from build123d import *

# Parameters (mm, degrees)
EXTRUDE_1_DEPTH           = 4
HOLE_WIZARD_1_D           = 3.4
HOLE_WIZARD_1_CBORE_D     = 6.5
HOLE_WIZARD_1_CBORE_DEPTH = 3.4
HOLE_WIZARD_M3_1_D        = 2.5
HOLE_WIZARD_M4_1_D        = 3.3
CHAMFER_1_SIZE            = 0.5


with BuildPart() as part:
    # 草图1 → 凸台-拉伸1 (new, symmetric)
    with BuildSketch(Plane(origin=(0, 0, 0), x_dir=(0, 0, -1), z_dir=(1, 0, 0))):
        with BuildLine():
            Line((20.5, -5), (-20.5, -5))
            ThreePointArc((-20.5, -5), (-25.5, 0), (-20.5, 5))
            Line((-20.5, 5), (20.5, 5))
            ThreePointArc((20.5, 5), (25.5, 0), (20.5, -5))
        make_face()
    extrude(amount=EXTRUDE_1_DEPTH, both=True)

    # 打孔尺寸(%根据)内六角圆柱头螺钉的类型1 (through all)
    with Locations(Plane(origin=(4, 0, 0), x_dir=(0, 0, -1), z_dir=(1, 0, 0))):
        with Locations((-20.5, 0)):
            CounterBoreHole(HOLE_WIZARD_1_D / 2, HOLE_WIZARD_1_CBORE_D / 2, HOLE_WIZARD_1_CBORE_DEPTH)

    # M3 螺纹孔1 (through all)
    with Locations(Plane(origin=(4, 0, 0), x_dir=(0, 0, -1), z_dir=(1, 0, 0))):
        with Locations((-4.5, 0)):
            Hole(HOLE_WIZARD_M3_1_D / 2)

    # M4 螺纹孔1 (through all)
    with Locations(Plane(origin=(4, 0, 0), x_dir=(0, 0, -1), z_dir=(1, 0, 0))):
        with Locations((20.5, 0)):
            Hole(HOLE_WIZARD_M4_1_D / 2)

    # 倒角1
    chamfer_1_edges = [part.edges().sort_by_distance(p)[0] for p in [
        (4, 0, 25.5),
        (4, -5, 0),
        (4, 0, -25.5),
        (-4, -5, 0),
        (-4, 0, 25.5),
        (-4, 5, 0),
        (-4, 0, -25.5),
        (4, 5, 0),
    ]]
    chamfer(chamfer_1_edges, length=CHAMFER_1_SIZE)


solid = part.part
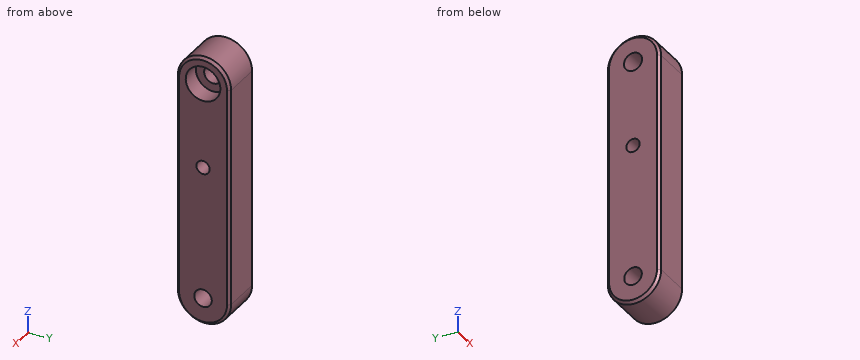
Source: CAD feature listing. Evaluate the final solid. Frame: model axes, mm. Give positions to 0.01 mm unless a question says otherwise; leave off trailing zeros. Order: outer loops, then holes, each group sorted by start corner. A loop starts at its lowest first (then second) coordinate and runs counter-clockwise, first axis right, second up. Notation, with made-up numbers: (-15.5, -26.75) -> (15.5, -26.75) arc R6 cw to (15.5, -16.75) -> close; hole circle Ø11 at (-25, 14). An arc over 180 degrees is marked (long way). Write item = value, one per line.
Q1. Cut plane A-A, the plane y = 0. Output: boundary loops of the cut face in (x, z).
Data:
outline = (-4, -25) -> (-3.5, -25.5) -> (3.5, -25.5) -> (4, -25) -> (4, -22.15) -> (-4, -22.15) -> close; (-4, -18.85) -> (4, -18.85) -> (4, 3.25) -> (-4, 3.25) -> close; (-4, 5.75) -> (4, 5.75) -> (4, 17.25) -> (0.6, 17.25) -> (0.6, 18.8) -> (-4, 18.8) -> close; (-4, 22.2) -> (0.6, 22.2) -> (0.6, 23.75) -> (4, 23.75) -> (4, 25) -> (3.5, 25.5) -> (-3.5, 25.5) -> (-4, 25) -> close
Q2. Cut plane D-D, the plane z = -20. Output: boundary loops of the cut face in (x, y), and give its area (3 significant figures).
Data:
outline = (-4, -4.5) -> (-3.5, -5) -> (3.5, -5) -> (4, -4.5) -> (4, -1.57) -> (-4, -1.57) -> close; (-4, 1.57) -> (4, 1.57) -> (4, 4.5) -> (3.5, 5) -> (-3.5, 5) -> (-4, 4.5) -> close
area = 54.3 mm^2
Q3. Cut plane B-B, the plane x = 2.5. Output: boundary loops of the cut face in (y, z).
Data:
outline = (-5, -20.5) arc R5 ccw to (5, -20.5) -> (5, 20.5) arc R5 ccw to (-5, 20.5) -> close; hole circle Ø6.5 at (0, 20.5); hole circle Ø3.3 at (0, -20.5); hole circle Ø2.5 at (0, 4.5)
Q4. Material intervals for line 1 (Y direction, x = -1.75, z = -20.5); line 2 (Y direction, x = -0.9, z = 20.5); line 3 (Z direction, x = 3.5, y = -0.75), sorted ascending. Write a range as from..to.
Data:
line_1 = -5..-1.65, 1.65..5
line_2 = -5..-1.7, 1.7..5
line_3 = -25.44..-21.97, -19.03..3.5, 5.5..17.34, 23.66..25.44
Q5. Cut plane C-C, the plane z = 4.5. Output: boundary loops of the cut face in (x, y), and give its area (3 significant figures).
Data:
outline = (-4, -4.5) -> (-3.5, -5) -> (3.5, -5) -> (4, -4.5) -> (4, -1.25) -> (-4, -1.25) -> close; (-4, 1.25) -> (4, 1.25) -> (4, 4.5) -> (3.5, 5) -> (-3.5, 5) -> (-4, 4.5) -> close
area = 59.5 mm^2
